from build123d import *

# Parameters (mm, degrees)
SKETCH1_W           = 40
SKETCH1_H           = 80
BOSS_EXTRUDE1_DEPTH = 2
SKETCH2_R           = 2.5
CUT_EXTRUDE1_DEPTH  = 10
CUT_EXTRUDE2_DEPTH  = 10


with BuildPart() as part:
    # Sketch1 → Boss-Extrude1 (new body)
    with BuildSketch(Plane(origin=(0, 0, 0), x_dir=(1, 0, 0), z_dir=(0, 1, 0))):
        Rectangle(SKETCH1_W, SKETCH1_H)
    extrude(amount=BOSS_EXTRUDE1_DEPTH)

    # Sketch2 → Cut-Extrude1 (cut)
    with BuildSketch(Plane.XZ):
        with Locations(Location((8, -20, 0), (0, 0, 270))):
            Circle(SKETCH2_R)
        with Locations(Location((-8, -20, 0), (0, 0, 270))):
            Circle(SKETCH2_R)
    extrude(amount=-CUT_EXTRUDE1_DEPTH, mode=Mode.SUBTRACT)

    # Sketch3 → Cut-Extrude2 (cut)
    with BuildSketch(Plane(origin=(0, 2, 0), x_dir=(1, 0, 0), z_dir=(0, 1, 0))):
        Polygon((-20, -40), (-12.784626592, -28.891322442), (-10.73702175, -35.778720546), (-6.263478534, -28.891322442), (-4.459373627, -34.959675311), (0.603406691, -25.613003955), (4.154649825, -34.959675311), (10.180946182, -29.559865215), (12.65531235, -34.959675311), (16.161083178, -33.353218681), (20, -40), align=None)
    extrude(amount=-CUT_EXTRUDE2_DEPTH, mode=Mode.SUBTRACT)


solid = part.part
The model under review builds one solid part; all positions refer to its coordinate system, in mm. A direction names the side the tool comes from. Coordinates: 2 decimals unless noted, no trailing zeros. Write each loop counter-clockwise with the first axis right and the second up, starting at its lowest first coordinate (ties: lowest second). Pieces come first, ordered by that corner, then holes. Notation, with made-up numbers: M 34,12.25 L 93,12.25 A8 cw 93,25.25 Z; hole C -34.5,-16 d8. An arc over 180 degrees is marked long. Put each result on its own line as item: value.
1) Add section A-A on z = -20. Give the boundary of the cut face in (x, y), then the cut area to 3 significant figures.
Computed:
outline: M -20,0 L -10.5,0 L -10.5,2 L -20,2 Z; M -5.5,0 L 5.5,0 L 5.5,2 L -5.5,2 Z; M 10.5,0 L 20,0 L 20,2 L 10.5,2 Z
area: 60.0 mm2
2) Draft analysis for pull direction Z (two halves, no side actions). For faces 1 (the flat face through (-1.963, 1.014, 30.352)), 2 (the cylindrical face through (-9.5, 1, -18)), 3 (the flat face through (-20, 1, 1)), state which applies: released by +Z, released by -Z, zero draft, split by the parting line, or undercut.
Computed:
face 1: released by +Z
face 2: undercut
face 3: zero draft
3) Wall thickness on probe 1 along X at (y, z) = (1.5, -20); probe 2 along X at (y, z) = (0.15, -21); probe 3 along X at (y, z) = (0.65, 31): over which ranges is each line inside the solid? List them lowest first. Write a range as [from, to].
Computed:
probe 1: x = [-20, -10.5], [-5.5, 5.5], [10.5, 20]
probe 2: x = [-20, -10.29], [-5.71, 5.71], [10.29, 20]
probe 3: x = [-20, -14.15], [-12.16, -7.63], [-5.64, -2.31], [2.65, 8.57], [10.84, 20]
4) For faces 4 (the flat face through (-11.775, 1.014, 32.287)), 5 (the cylindrical face through (6.5, 1, -18)), list the 3-axis set-ups (+Z, -Z, +X, -X, +Y, -Y) from which the entire face can be reached by the end or side of a thin tool; tool diameter is ignored.
Computed:
face 4: +Z, +Y, -Y
face 5: +Y, -Y
5) Add section D-D on x = 8. Give the boundary of the cut face in (y, z).
Computed:
outline: M 0,-40 L 2,-40 L 2,-22.5 L 0,-22.5 Z; M 0,-17.5 L 2,-17.5 L 2,31.51 L 0,31.51 Z
6) Add section B-B on y = 0.7. Give the boundary of the cut face in (x, z).
Computed:
outline: M -20,-40 L 20,-40 L 20,40 L 16.16,33.35 L 12.66,34.96 L 10.18,29.56 L 4.15,34.96 L 0.6,25.61 L -4.46,34.96 L -6.26,28.89 L -10.74,35.78 L -12.78,28.89 L -20,40 Z; hole C -8,-20 d5; hole C 8,-20 d5
7) Add section C-C on x = -7. Give the boundary of the cut face in (y, z), then the cut area to 3 significant figures.
Computed:
outline: M 0,-40 L 2,-40 L 2,-22.29 L 0,-22.29 Z; M 0,-17.71 L 2,-17.71 L 2,30.03 L 0,30.03 Z
area: 131 mm2
